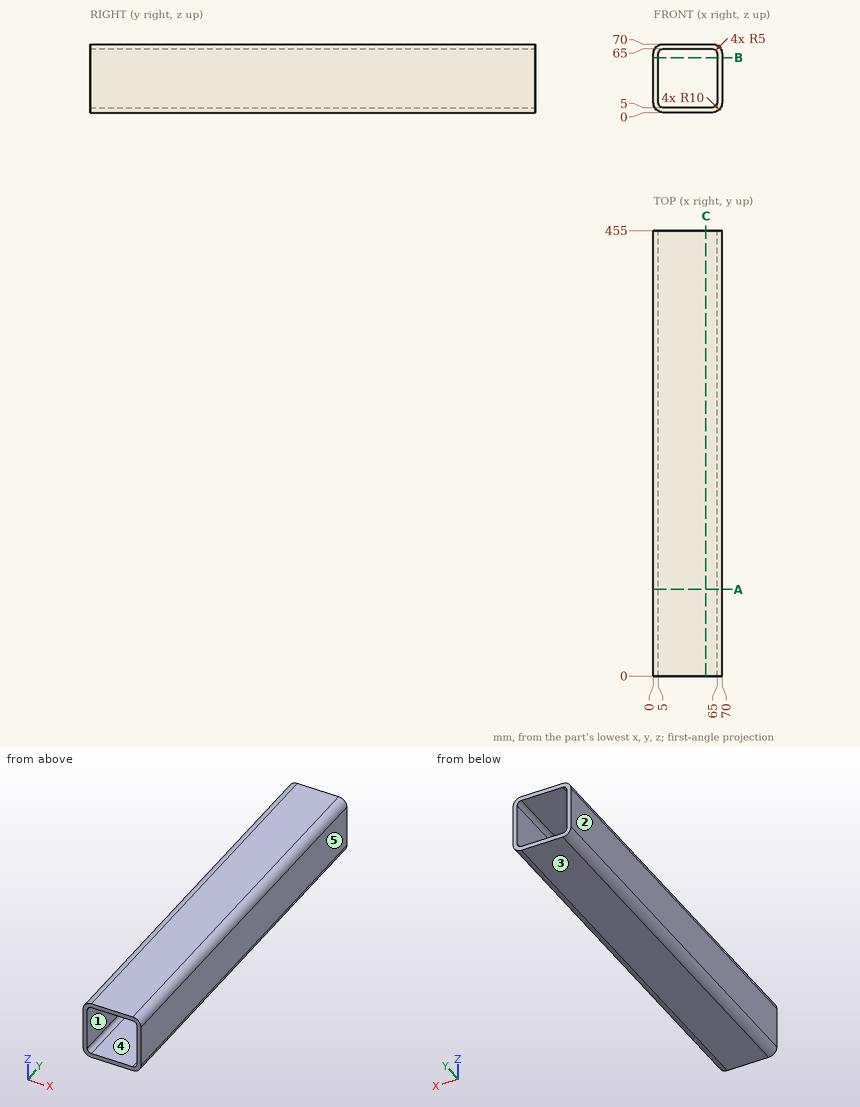
Geometry check sheet. Reference: drawing and pictorial views, mm from the part's lowest x, y, z. A direction names the side the tool comes from. Give positions to 0.01 mm unless a question says otherwise; leave off trailing zeros. Write each loop counter-clockwise with the first axis right and the second up, starting at its lowest first coordinate (ties: lowest second). Pieces come first, ordered by that corner, then holes. Notation, with made-up numbers: M 38.5,55.5 L 96.5,55.5 A21 cw 96.5,83.5 Z; hole C -18.5,59.5 d8. An arc over 180 degrees is marked long. Put each result on its own line as item: value. Start each with the question number.
1. Section check B-B (z = 56). Record the cut outline in (x, y).
2. Section check C-C (x = 53.5). Record the cut outline in (y, z), and give its area (3 significant figures).
3. Scan line: line 1 along Z through (x, y) = (46.5, 194). Record every from-to range of solid material in increasing order. Write a range as [from, to].
4. Set-up check for the marked faces 1 and 2: record each of +Z, -Z, +X, -X, +Y, -Y from which the full face is reachable in a straight line by a thin tool's end or side.
5. Draft check along X on the marked faces 3, 4 and 5. Enter one of: +X half, -X half, draft (parallel to the pull), parting line (faces both ways), or undercut.
6. Section check A-A (y = 88.5). Record the cut outline in (x, z).
Answer list:
1. outline: M 0,0 L 5,0 L 5,455 L 0,455 Z; M 65,0 L 70,0 L 70,455 L 65,455 Z
2. outline: M 0,0 L 455,0 L 455,5 L 0,5 Z; M 0,65 L 455,65 L 455,70 L 0,70 Z
2. area: 4,550 mm2
3. line 1: [0, 5], [65, 70]
4. face 1: +Y, -Y
4. face 2: +Z, -Z, -X, +Y, -Y
5. face 3: draft
5. face 4: undercut
5. face 5: +X half
6. outline: M 0,10 A10 ccw 10,0 L 60,0 A10 ccw 70,10 L 70,60 A10 ccw 60,70 L 10,70 A10 ccw 0,60 Z; hole M 5,10 A5 ccw 10,5 L 60,5 A5 ccw 65,10 L 65,60 A5 ccw 60,65 L 10,65 A5 ccw 5,60 Z
